Source: CAD feature listing. Evaluate the final solid. Frame: model axes, mm. Face numbers are marked on the shaded views. A direction names the side the tool comes from. Coordinates: 2 decimals unless noted, no trailing zeros. Order: outer loops, then holes, each group sorted by start corner. A loop starts at its lowest first (then second) coordinate and runs counter-clockwise, first axis right, second up.
```python
from build123d import *

# Parameters (mm, degrees)
SKETCH1_R           = 9.525
BOSS_EXTRUDE1_DEPTH = 9.525
SKETCH2_R           = 3.175
BOSS_EXTRUDE2_DEPTH = 4.7625
BOSS_EXTRUDE3_START = 4.7625
SKETCH3_R           = 3.175
BOSS_EXTRUDE3_DEPTH = 4.7625
SKETCH4_R           = 3.175
CUT_EXTRUDE1_DEPTH  = 20.636290542


with BuildPart() as part:
    # Sketch1 → Boss-Extrude1 (new body)
    with BuildSketch(Plane.XY):
        Circle(SKETCH1_R)
    extrude(amount=-BOSS_EXTRUDE1_DEPTH)

    # Sketch2 → Boss-Extrude2 (add)
    with BuildSketch(Plane.XY):
        with Locations(Location((0, 0, 0), (0, 0, 180))):
            Circle(SKETCH2_R)
    extrude(amount=BOSS_EXTRUDE2_DEPTH)

    # Sketch3 → Boss-Extrude3 (add)
    with BuildSketch(Plane(origin=(0, 0, -9.525), x_dir=(-1, 0, 0), z_dir=(0, 0, -1)).offset(BOSS_EXTRUDE3_START)):
        Circle(SKETCH3_R)
    extrude(amount=-BOSS_EXTRUDE3_DEPTH)

    # Sketch4 → Cut-Extrude1 (cut, through all)
    with BuildSketch(Plane(origin=(0, 0, 0), x_dir=(0, 0, -1), z_dir=(1, 0, 0))):
        with Locations((4.7625, 0)):
            Circle(SKETCH4_R)
    extrude(amount=CUT_EXTRUDE1_DEPTH, mode=Mode.SUBTRACT)


solid = part.part
```
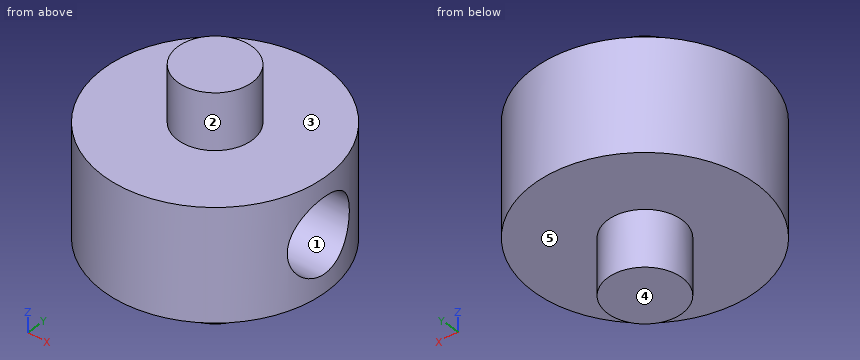
1. Pin query (flat end, axial travel): P1, Ø1.5, axis at y = 5.5, z = -4, coming from the -X side; P2, Ø3, axis at x = -7, y = -5.5, coming from the +Z side; P3, Ø2, axis at y = -6.5, z = -7.5, coming from the +X side. Return the tip coordinate at first contact, or that it passes through.
Findings:
P1: stops at x = -8.26
P2: stops at z = 0
P3: stops at x = 7.78
2. Section query D-D on x = -8.5. Return loops of the section in (y, z) (3 decimals).
Findings:
outline: (-4.298, -9.525) - (4.298, -9.525) - (4.298, 0) - (-4.298, 0) - close
3. Access query for the marked faces 4 and 5. Directions: +Z, -Z, +X, -X, +Y, -Y. A direction counts if a zero-diameter tool reaches every point of the face in a straight line with its end or side. Return the directions, or none.
Findings:
face 4: -Z, +X, -X, +Y, -Y
face 5: -Z
4. Section query C-C on z = -10.25. Return loops of the section in (x, y) (3 decimals), plus the area to 3 significant figures.
Findings:
outline: circle Ø6.35 at (0, 0)
area: 31.7 mm2
5. Section query A-A on y = 0. Return loops of the section in (x, z) (1 decimal).
Findings:
outline: (-9.5, -9.5) - (-3.2, -9.5) - (-3.2, -14.3) - (3.2, -14.3) - (3.2, -9.5) - (9.5, -9.5) - (9.5, -7.9) - (0, -7.9) - (0, -1.6) - (9.5, -1.6) - (9.5, 0) - (3.2, 0) - (3.2, 4.8) - (-3.2, 4.8) - (-3.2, 0) - (-9.5, 0) - close
6. Draft query along Y for the marked faces 1, 2 and 3. Return one class per face: released by +Y, released by -Y, zero draft, split by the parting line, or undercut.
Findings:
face 1: undercut
face 2: split by the parting line
face 3: zero draft
7. Ray query, line 1 (Z direction, x = 5, y = 0) (1 decimal); line 2 (X direction, y = 0.25, z = -5.5); line 3 (Z direction, x = 6, y = -7) (3 decimals). Return the intervals inside material, ascending.
Findings:
line 1: z = -9.5 to -7.9, -1.6 to 0
line 2: x = -9.52 to 0
line 3: z = -9.525 to 0
